Check sheet for the modelled part. Datum: model origin and axes. Units: mm. Round coordinates to 2 decimals unless told otherwise and drop trailing zeros. Write each loop counter-clockwise with the first axis right and the second up, starting at its lowest first coordinate (ties: lowest second). Pieces come first, ordered by that corner, then holes. Notation, with made-up numbers: M 13.5,-35 L 61.5,-35 A26 cw 61.5,-5 Z; hole C 56,-3.75 d8. An arc over 180 degrees is marked long. Put each result on its own line as item: value.
```python
from build123d import *

# Parameters (mm, degrees)
SKETCH1_R           = 6.35
BOSS_EXTRUDE1_DEPTH = 10.16
SCALE1_SCALE        = 2


with BuildPart() as part:
    # Sketch1 → Boss-Extrude1 (new body)
    with BuildSketch(Plane.XY):
        Polygon((6.73459618, 5.803215857), (-1.658434266, 8.733939305), (-8.393030446, 2.930723448), (-6.73459618, -5.803215857), (1.658434266, -8.733939305), (8.393030446, -2.930723448), align=None)
        Circle(SKETCH1_R, mode=Mode.SUBTRACT)
    extrude(amount=BOSS_EXTRUDE1_DEPTH)


with BuildPart() as part_1:
    # Scale1: scaled about (0, 0, 0)
    add(part.part.scale(SCALE1_SCALE))


solid = part_1.part
```
1. Scan lines: probe 1 along X at (y, z) = (-1, 15.25); probe 2 along X at (y, z) = (7, 9); probe 3 along Y at (x, z) = (0, 5.5). Record each from-to range of solid material in increasing order.
Computed values:
probe 1: x = -15.48 to -12.66, 12.66 to 15.86
probe 2: x = -15.46 to -10.6, 10.6 to 14.34
probe 3: y = -16.31 to -12.7, 12.7 to 16.31
2. Release check for a two-part mould opening along X. For faces 1 (the flat face through (0, -13, 20.32)), 2 (the cylindrical face through (-2.75, -12.4, 10.02)), 3 (the flat face through (-9.957, 11.746, 10.018)) record: +X half, -X half, draft (parallel to the pull), parting line (faces both ways), or undercut.
Computed values:
face 1: draft
face 2: undercut
face 3: -X half
3. Depth check by flat-ended pin: pin 1 Ø1.5 at (x, z) = (-8.5, 17) entering from +Y; pin 2 Ø8 at (x, z) = (-8, 3) entering from -Y; pin 3 Ø1 at (y, z) = (-12.5, 16.5) entering from +X. Enter the tip coordinate at first touch or a pass-through.
Computed values:
pin 1: stops at y = 13.65
pin 2: stops at y = -14.91
pin 3: stops at x = 9.66
4. Cross-section at A-A (z = 10.5). Enter the section's corners in (x, y), then the cut area to 3 significant figures.
Computed values:
outline: M -16.79,5.86 L -13.47,-11.61 L 3.32,-17.47 L 16.79,-5.86 L 13.47,11.61 L -3.32,17.47 Z; hole C 0,0 d25.4
area: 315 mm2
5. Cross-section at B-B (x = -5.5). Enter the section's corners in (y, z), then the cut area to 3 significant figures.
Computed values:
outline: M -14.39,0 L -11.45,0 L -11.45,20.32 L -14.39,20.32 Z; M 11.45,0 L 15.59,0 L 15.59,20.32 L 11.45,20.32 Z
area: 144 mm2
6. Cross-section at D-D (x = 14). Enter the section's corners in (y, z).
Computed values:
outline: M -8.26,0 L 8.81,0 L 8.81,20.32 L -8.26,20.32 Z
7. Cross-section at C-C (y = -9.5). Enter the section's corners in (x, z).
Computed values:
outline: M -13.87,0 L -8.43,0 L -8.43,20.32 L -13.87,20.32 Z; M 8.43,0 L 12.56,0 L 12.56,20.32 L 8.43,20.32 Z
